Build history of the part. All positions in model axes, mm. Coordinates: 2 decimals unless noted, no trailing zeros. Write each loop counter-clockwise with the first axis right and the second up, starting at its lowest first coordinate (ties: lowest second). Pieces come first, ordered by that corner, then holes.
```python
from build123d import *

# Parameters (mm, degrees)
EXTRUDE_1_DEPTH     = 7
SKETCH_2_R          = 1.55
CUT_EXTRUDE_1_DEPTH = 7


with BuildPart() as part:
    # 草图1 → 凸台-拉伸1 (new body)
    with BuildSketch(Plane.XY):
        with BuildLine():
            Line((8.5, 8.5), (-8.5, 8.5))
            Line((-8.5, 8.5), (-8.5, 0.5))
            Line((-8.5, 0.5), (-6.982120022, 0.5))
            ThreePointArc((-6.982120022, 0.5), (0, 7), (6.982120022, 0.5))
            Line((6.982120022, 0.5), (8.5, 0.5))
            Line((8.5, 0.5), (8.5, 8.5))
        make_face()
    extrude(amount=EXTRUDE_1_DEPTH)

    # 草图2 → 切除-拉伸1 (cut)
    with BuildSketch(Plane(origin=(0, 8.5, 0), x_dir=(1, 0, 0), z_dir=(0, 1, 0))):
        with Locations(Location((0, -3.5, 0), (0, 0, 270))):
            Circle(SKETCH_2_R)
    extrude(amount=-CUT_EXTRUDE_1_DEPTH, mode=Mode.SUBTRACT)


solid = part.part
```
1. Probe line 1 along X through (y, z) = (7.95, 3.5); line 2 along Z through (x, y) = (0, 7.85); line 3 along X through (y, z) = (3.75, 4.5). List the from-to ranges inside material, lowest first.
Computed values:
line 1: x = -8.5 to -1.55, 1.55 to 8.5
line 2: z = 0 to 1.95, 5.05 to 7
line 3: x = -8.5 to -5.91, 5.91 to 8.5
2. Saw through at A-A on z = 3.5. List the corners of the cut face in (x, y).
Computed values:
outline: (-8.5, 0.5) - (-6.98, 0.5) arc R7 cw to (-1.55, 6.83) - (-1.55, 8.5) - (-8.5, 8.5) - close; (1.55, 6.83) arc R7 cw to (6.98, 0.5) - (8.5, 0.5) - (8.5, 8.5) - (1.55, 8.5) - close
3. Saw through at C-C on y = 1.5. List the corners of the cut face in (x, z).
Computed values:
outline: (-8.5, 0) - (-6.84, 0) - (-6.84, 7) - (-8.5, 7) - close; (6.84, 0) - (8.5, 0) - (8.5, 7) - (6.84, 7) - close
4. Saw through at B-B on x = 0. List the corners of the cut face in (y, z), plus the area to 3 significant figures.
Computed values:
outline: (7, 0) - (8.5, 0) - (8.5, 1.95) - (7, 1.95) - close; (7, 5.05) - (8.5, 5.05) - (8.5, 7) - (7, 7) - close
area: 5.85 mm2
5. Saw through at D-D on z = 1.75. List the corners of the cut face in (x, y).
Computed values:
outline: (-8.5, 0.5) - (-6.98, 0.5) arc R7 cw to (6.98, 0.5) - (8.5, 0.5) - (8.5, 8.5) - (-8.5, 8.5) - close
6. Mould opens along Z. For faces 1 (the face through (8.5, 4, 3)), 2 (the face through (1.537, 7.675, 3.298)), 3 (the face through (-0.1, 7.2, 0)), 4 (the face through (-0.1, 7.2, 7)) say: +Z half, -Z half, draft (parallel to the pull), parting line (faces both ways), or undercut.
Computed values:
face 1: draft
face 2: undercut
face 3: -Z half
face 4: +Z half
